```python
from build123d import *

# Parameters (mm, degrees)
BASE_PLATE_SKETCH_W    = 74
BASE_PLATE_SKETCH_H    = 76
BASE_PLATE_DEPTH       = 10
FLANGE_EAR_A_SKETCH_R  = 5
FLANGE_EAR_A_DEPTH     = 10
FLANGE_START           = -10
FLANGE_EAR_B_SKETCH_R  = 5
FLANGE_EAR_B_DEPTH     = 10
TRANSITION_BOSS_DEPTH  = 10
HUB_40_SKETCH_R        = 20
HUB_40_DEPTH           = 40
SHAFT_26_SKETCH_R      = 13
SHAFT_26_DEPTH         = 100
SHAFT_START            = -60
SHAFT_FLAT_CUT_DEPTH   = 60
SHAFT_EDGE_FILLET_R3_R = 3


with BuildPart() as part:
    # Base Plate Sketch → Base Plate (new body)
    with BuildSketch(Plane.XY):
        Rectangle(BASE_PLATE_SKETCH_W, BASE_PLATE_SKETCH_H)
    extrude(amount=BASE_PLATE_DEPTH)

    # Flange Ear A Sketch → Flange Ear A (add)
    with BuildSketch(Plane(origin=(0, 38, 0), x_dir=(1, 0, 0), z_dir=(0, 1, 0))):
        with BuildLine():
            Line((-37, -10), (-13.060137394, -52.377859531))
            ThreePointArc((-13.060137394, -52.377859531), (0, -60), (13.060137394, -52.377859531))
            Line((13.060137394, -52.377859531), (37, -10))
            Line((37, -10), (-37, -10))
        make_face()
        with Locations(Location((0, -45, 0), (0, 0, 270))):
            Circle(FLANGE_EAR_A_SKETCH_R, mode=Mode.SUBTRACT)
    extrude(amount=-FLANGE_EAR_A_DEPTH)

    # Flange Ear B Sketch → Flange Ear B (add)
    with BuildSketch(Plane.XZ.offset(38).offset(FLANGE_START)):
        with BuildLine():
            Line((-37, 10), (-13.060137394, 52.377859531))
            ThreePointArc((-13.060137394, 52.377859531), (0, 60), (13.060137394, 52.377859531))
            Line((13.060137394, 52.377859531), (37, 10))
            Line((37, 10), (-37, 10))
        make_face()
        with Locations(Location((0, 45, 0), (0, 0, 90))):
            Circle(FLANGE_EAR_B_SKETCH_R, mode=Mode.SUBTRACT)
    extrude(amount=FLANGE_EAR_B_DEPTH)

    # Transition Boss Sketch → Transition Boss (add)
    with BuildSketch(Plane(origin=(0, 0, 0), x_dir=(-1, 0, 0), z_dir=(0, 0, -1))):
        with BuildLine():
            Line((19.921474427, 22.430667771), (-20.596234674, 21.812728331))
            ThreePointArc((-20.596234674, 21.812728331), (-22.10962434, 20.277191904), (-23.508824666, 18.636930081))
            ThreePointArc((-23.508824666, 18.636930081), (-30, 0), (-23.508824666, -18.636930081))
            ThreePointArc((-23.508824666, -18.636930081), (-22.10962434, -20.277191904), (-20.596234674, -21.812728331))
            Line((-20.596234674, -21.812728331), (19.921474427, -22.430667771))
            ThreePointArc((19.921474427, -22.430667771), (21.797840059, -20.611990897), (23.508824666, -18.636930081))
            ThreePointArc((23.508824666, -18.636930081), (30, 0), (23.508824666, 18.636930081))
            ThreePointArc((23.508824666, 18.636930081), (21.797840059, 20.611990897), (19.921474427, 22.430667771))
        make_face()
    extrude(amount=TRANSITION_BOSS_DEPTH)

    # Hub _40 Sketch → Hub _40 (add)
    with BuildSketch(Plane(origin=(0, 0, -10), x_dir=(-1, 0, 0), z_dir=(0, 0, -1))):
        Circle(HUB_40_SKETCH_R)
    extrude(amount=HUB_40_DEPTH)

    # Shaft _26 Sketch → Shaft _26 (add)
    with BuildSketch(Plane(origin=(0, 0, -50), x_dir=(-1, 0, 0), z_dir=(0, 0, -1))):
        Circle(SHAFT_26_SKETCH_R)
    extrude(amount=SHAFT_26_DEPTH)

    # Shaft Flat Sketch → Shaft Flat Cut (cut)
    with BuildSketch(Plane(origin=(0, 0, -150), x_dir=(-1, 0, 0), z_dir=(0, 0, -1)).offset(SHAFT_START)):
        with BuildLine():
            Line((-10.246950766, 8), (10.246950766, 8))
            ThreePointArc((10.246950766, 8), (0, 13), (-10.246950766, 8))
        make_face()
    extrude(amount=SHAFT_FLAT_CUT_DEPTH, mode=Mode.SUBTRACT)

    # Shaft Edge Fillet R3
    shaft_edge_fillet_r3_edges = [part.edges().sort_by_distance(p)[0] for p in [
        (4.230226947, -12.292484695, -150),
    ]]
    fillet(shaft_edge_fillet_r3_edges, radius=SHAFT_EDGE_FILLET_R3_R)


solid = part.part
```
CAD build for the part. Positions are in the model's coordinates, mm. A direction names the side the tool comes from. Round coordinates to 2 decimals unless told otherwise and drop trailing zeros. Order: outer loops, then holes, each group sorted by start corner. A loop starts at its lowest first (then second) coordinate and runs counter-clockwise, first axis right, second up. Notation, with made-up numbers: (55.5, -26.75) - (107.5, -26.75) arc R18 ccw to (107.5, -13.75) - close; hole circle Ø2 at (-13.5, -23). An arc over 180 degrees is marked (long way). Answer in a Markdown table with one row per item. Add a question column.
(1) Band-saw the part on C-C on z = 45. List the corners of the cut face in (x, y).
(2) 3-axis set-ups, long thin cutter, end or side, ignore diameter. For faces 1 (the face through (20.4, 0.3, -10)), 2 (the face through (-1, 0, 10)), 3 (the face through (0, 10, -90)): which of +Z, -Z, +X, -X, +Y, -Y reach the whole face in a straight line?
(3) Band-saw the part on B-B on x = 0. Count the separate pieces of the cut face and the enclosed holes in it, and give its area (3 significant figures).
(4) Probe L1, parallel to Y at x = -21, z = 27; L2, parallel to Z at x = 34, y = -17; L3, parallel to Z at x = 17, y = 1. List the from-to ranges inside material, lowest first. Write a range as [from, to].
(5) Band-saw the part on D-D on z = -44. List the corners of the cut face in (x, y), and give its area (3 significant figures).
(6) Band-saw the part on A-A on y = 0. List the corners of the cut face in (x, z).
(7) Drop flat-ended pins along their axis: pin 1 Ø4 at (x, y) = (-2, 10.5) entering from -Z; pin 2 Ø4 at (y, z) = (3.5, -114.5) entering from -X; pin 3 Ø1.5 at (x, z) = (-2, -34.5) entering from -Y. Give the stop position or say it passes through.
Data:
| question | item | result |
|---|---|---|
| 1 | outline | (-17.23, -38) - (-5, -38) - (-5, -28) - (-17.23, -28) - close; (-17.23, 28) - (-5, 28) - (-5, 38) - (-17.23, 38) - close; (5, -38) - (17.23, -38) - (17.23, -28) - (5, -28) - close; (5, 28) - (17.23, 28) - (17.23, 38) - (5, 38) - close |
| 2 | face 1 | -Z |
| 2 | face 2 | +Z, +X, -X |
| 2 | face 3 | -Z, +X, -X, +Y |
| 3 | separate pieces | 3 |
| 3 | enclosed holes | 0 |
| 3 | area | 5,900 mm^2 |
| 4 | L1 | y = [-38, -28], [28, 38] |
| 4 | L2 | z = [0, 10] |
| 4 | L3 | z = [-50, 10] |
| 5 | outline | circle Ø40 at (0, 0) |
| 5 | area | 1,260 mm^2 |
| 6 | outline | (-37, 0) - (-30, 0) - (-30, -10) - (-20, -10) - (-20, -50) - (-13, -50) - (-13, -147) arc R3 ccw to (-10, -150) - (10, -150) arc R3 ccw to (13, -147) - (13, -50) - (20, -50) - (20, -10) - (30, -10) - (30, 0) - (37, 0) - (37, 10) - (-37, 10) - close |
| 7 | pin 1 | stops at z = -90 |
| 7 | pin 2 | stops at x = -12.91 |
| 7 | pin 3 | stops at y = -19.96 |
